CAD build for the part. Positions are in the model's coordinates, mm. A direction names the side the tool comes from. Coordinates: 2 decimals unless noted, no trailing zeros. Loops run counter-clockwise (first coordinate to the right, second up) from the corner with the lowest first, then second, coordinate; pieces in that order, holes last. Notation, with made-up numbers: (48.25, 33) -> (90.25, 33) arc R25 ccw to (90.25, 46) -> close; hole circle Ø9 at (-2, 4.25). An arc over 180 degrees is marked (long way). Answer as CSV lines item,"result". Start each with the question number.
from build123d import *

# Parameters (mm, degrees)
SKETCH1_W                                           = 60
SKETCH1_H                                           = 165
BOSS_EXTRUDE1_DEPTH                                 = 10
CBORE_FOR_M6_HEX_SOCKET_HEAD_CAP_SCREW1_D           = 6.6
CBORE_FOR_M6_HEX_SOCKET_HEAD_CAP_SCREW1_CBORE_D     = 11
CBORE_FOR_M6_HEX_SOCKET_HEAD_CAP_SCREW1_CBORE_DEPTH = 6.4
CBORE_FOR_M5_HEX_SOCKET_HEAD_CAP_SCREW2_D           = 5.5
CBORE_FOR_M5_HEX_SOCKET_HEAD_CAP_SCREW2_CBORE_D     = 10
CBORE_FOR_M5_HEX_SOCKET_HEAD_CAP_SCREW2_CBORE_DEPTH = 5.4
FILLET1_R                                           = 5


with BuildPart() as part:
    # Sketch1 → Boss-Extrude1 (new body)
    with BuildSketch(Plane.XY):
        Rectangle(SKETCH1_W, SKETCH1_H)
    extrude(amount=BOSS_EXTRUDE1_DEPTH)

    # CBORE for M6 Hex Socket Head Cap Screw1 (through all)
    with Locations(Plane.XY.offset(10)):
        with Locations((-10, 26), (10, 26), (10, -26), (-10, -26)):
            CounterBoreHole(CBORE_FOR_M6_HEX_SOCKET_HEAD_CAP_SCREW1_D / 2, CBORE_FOR_M6_HEX_SOCKET_HEAD_CAP_SCREW1_CBORE_D / 2, CBORE_FOR_M6_HEX_SOCKET_HEAD_CAP_SCREW1_CBORE_DEPTH)

    # CBORE for M5 Hex Socket Head Cap Screw2 (through all)
    with Locations(Plane.XY.offset(10)):
        with Locations((4.94295756, 76), (4.94295756, 44), (4.94295756, -44), (4.94295756, -76)):
            CounterBoreHole(CBORE_FOR_M5_HEX_SOCKET_HEAD_CAP_SCREW2_D / 2, CBORE_FOR_M5_HEX_SOCKET_HEAD_CAP_SCREW2_CBORE_D / 2, CBORE_FOR_M5_HEX_SOCKET_HEAD_CAP_SCREW2_CBORE_DEPTH)

    # Fillet1
    fillet1_edges = [part.edges().sort_by_distance(p)[0] for p in [
        (30, -82.5, 5),
        (-30, -82.5, 5),
        (-30, 82.5, 5),
        (30, 82.5, 5),
    ]]
    fillet(fillet1_edges, radius=FILLET1_R)


solid = part.part
Item 1: Saw through at C-C (y = 26). Write the cut outline in (x, z).
Item 2: Saw through at B-B (y = -44). Write the cut outline in (x, z), plus the area to 3 significant figures.
Item 3: Two-plate mould, pull along Y, no slides. Class faces 3 (the face through (0, -82.5, 5)), 4 (the face through (7.1, -78.2, 4.6)), 5 (the face through (30, -1, 5)): pulls with the +Y half, pulls with the -Y half, needs draft (parallel to the pull), parting line crosses it, or undercut.
Item 4: Which spindle directions (+Z, -Z, +X, -X, +Y, -Y) get a long thin tool onto all of the face, cutting with end or side? Do faces 1 (the face through (-7.043, 30.638, 6.845)), 2 (the face through (0, 1, 0)). Say none if no direction does.
Item 5: Saw through at A-A (x = -10). Write the cut outline in (y, z).
Item 6: Saw through at D-D (z = 2). Count the separate pieces of the cut face and the enclosed holes in it, plus the area to 3 significant figures.
Item 7: Wall check: probe 1 along Y at (x, z) = (-10, 5.25); probe 2 along Y at (x, z) = (-10, 1.25); probe 3 along X at (y, z) = (-23.5, 2). Give the ranges that are in metal, low to high.
Item 8: Flat gauge pins, fed straight in: pin 1 Ø5.5 at (x, y) = (11, 26) entering from +Z; pin 2 Ø8 at (x, y) = (15, 12) entering from -Z; pin 3 Ø3 at (x, y) = (4, -75) entering from +Z; pin 4 Ø5 at (x, y) = (4.94, -76) entering from -Z. Where does each tip first touch, or does it go through?
Geometry check:
1,outline,"(-30, 0) -> (-13.3, 0) -> (-13.3, 3.6) -> (-15.5, 3.6) -> (-15.5, 10) -> (-30, 10) -> close; (-6.7, 0) -> (6.7, 0) -> (6.7, 3.6) -> (4.5, 3.6) -> (4.5, 10) -> (-4.5, 10) -> (-4.5, 3.6) -> (-6.7, 3.6) -> close; (13.3, 0) -> (30, 0) -> (30, 10) -> (15.5, 10) -> (15.5, 3.6) -> (13.3, 3.6) -> close"
2,outline,"(-30, 0) -> (2.19, 0) -> (2.19, 4.6) -> (-0.06, 4.6) -> (-0.06, 10) -> (-30, 10) -> close; (7.69, 0) -> (30, 0) -> (30, 10) -> (9.94, 10) -> (9.94, 4.6) -> (7.69, 4.6) -> close"
2,area,"521 mm2"
3,face 3,"pulls with the -Y half"
3,face 4,"undercut"
3,face 5,"needs draft"
4,face 1,"+Z"
4,face 2,"-Z, +X, -X, +Y, -Y"
5,outline,"(-82.5, 0) -> (-29.3, 0) -> (-29.3, 3.6) -> (-31.5, 3.6) -> (-31.5, 10) -> (-82.5, 10) -> close; (-22.7, 0) -> (22.7, 0) -> (22.7, 3.6) -> (20.5, 3.6) -> (20.5, 10) -> (-20.5, 10) -> (-20.5, 3.6) -> (-22.7, 3.6) -> close; (29.3, 0) -> (82.5, 0) -> (82.5, 10) -> (31.5, 10) -> (31.5, 3.6) -> (29.3, 3.6) -> close"
6,separate pieces,"1"
6,enclosed holes,"8"
6,area,"9,650 mm2"
7,probe 1,"-82.5 to -31.5, -20.5 to 20.5, 31.5 to 82.5"
7,probe 2,"-82.5 to -29.3, -22.7 to 22.7, 29.3 to 82.5"
7,probe 3,"-30 to -12.15, -7.85 to 7.85, 12.15 to 30"
8,pin 1,"z = 3.6"
8,pin 2,"z = 0"
8,pin 3,"z = 4.6"
8,pin 4,"through"
